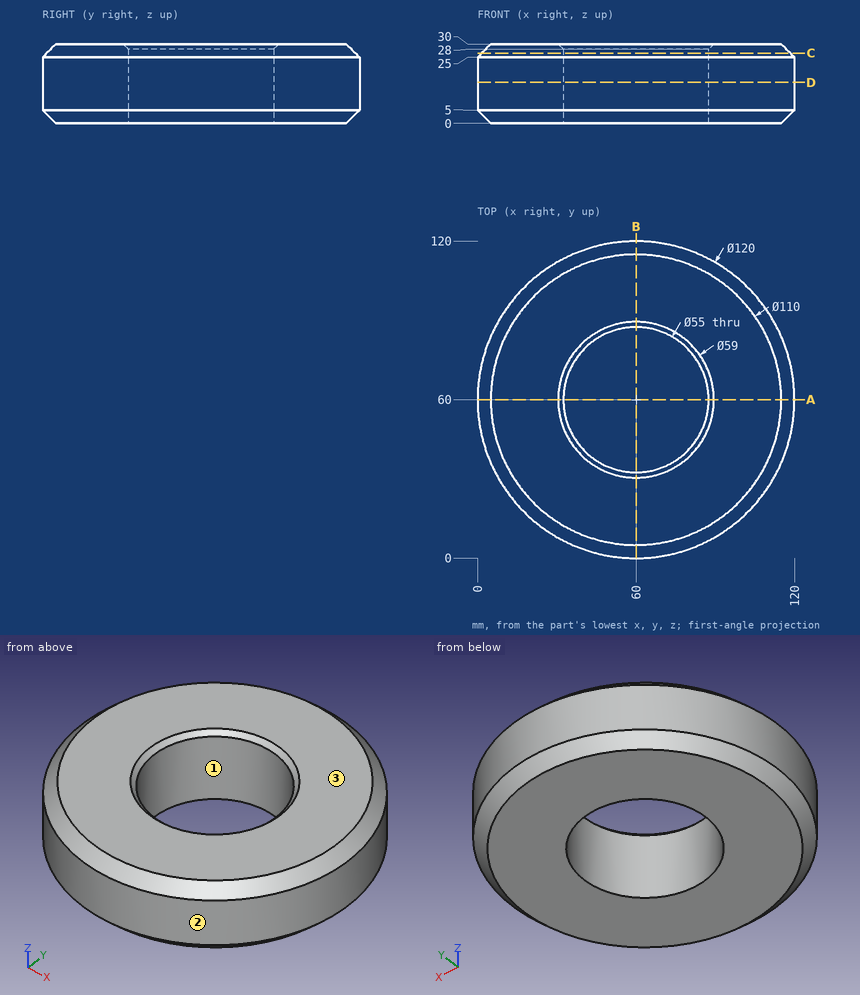
Answer from the drawing. Dimensions are ordinates in mm from the lowest x, y and z of the part. Coordinates: 2 decimals unless noted, no trailing zeros. Order: outer loops, then holes, each group sorted by start corner. A loop starts at its lowest first (then second) coordinate and runs counter-clockwise, first axis right, second up. Notation, with made-up numbers: (-2, 24.25) - (24, 24.25) arc R18 cw to (24, 58.25) - close; hole circle Ø7 at (28.25, 52.5). An arc over 180 degrees is marked (long way). Put each result on its own line as item: value. Start each with the question number.
1) Find section D-D (z = 15.5). Give the vertices of the cut face in (x, y).
2) For a pull along Y with two mould halves and no side action, classify the marked faces 1, 2 and 3 as released by +Y, released by -Y, zero draft, split by the parting line, or undercut.
3) Find the intervals of material crossed by line 1 (Y direction, x = 60, z = 12); line 2 (Y direction, x = 80.5, z = 2); line 3 (X direction, y = 47, z = 4.75), in increasing order. Write a range as from..to.
4) Find section A-A (y = 60). Give the vertices of the cut face in (x, z).
5) Flat-ended cylindrical pins translate along their axes: pin 1 (1 mm diameter, centred on x = 68, z = 19, fed in from +Y); pin 2 (10 mm diameter, centred on y = 28.5, z = 14.5, fed in from -X); pin 3 (2 mm diameter, centred on y = 37, z = 22.5, fed in from +X). Find the tip coordinate at first contact, or state that the pin passes through.
6) Find section C-C (z = 26.5). Give the vertices of the cut face in (x, y).
Results list:
1. outline: circle Ø120 at (60, 60); hole circle Ø55 at (60, 60)
2. face 1: undercut
2. face 2: split by the parting line
2. face 3: zero draft
3. line 1: y = 0..32.5, 87.5..120
3. line 2: y = 6.81..41.67, 78.33..113.19
3. line 3: x = 1.68..35.77, 84.23..118.32
4. outline: (0, 5) - (5, 0) - (32.5, 0) - (32.5, 28) - (30.5, 30) - (5, 30) - (0, 25) - close; (87.5, 0) - (115, 0) - (120, 5) - (120, 25) - (115, 30) - (89.5, 30) - (87.5, 28) - close
5. pin 1: stops at y = 119.53
5. pin 2: stops at x = 6.17
5. pin 3: stops at x = 115.82
6. outline: circle Ø117 at (60, 60); hole circle Ø55 at (60, 60)
